from build123d import *

# Parameters (mm, degrees)
BASE_BLOCK_70X40X40_DEPTH        = 40
BOTTOM_SLOT_SKETCH_W             = 24
BOTTOM_SLOT_SKETCH_H             = 14
BOTTOM_SLOT_DEPTH                = 35
BOTTOM_SLOT_EXTENSION_SKETCH_W   = 24
BOTTOM_SLOT_EXTENSION_SKETCH_H   = 14
BOTTOM_SLOT_EXTENSION_DEPTH      = 35
TOP_CHANNEL_SKETCH_W             = 14
TOP_CHANNEL_SKETCH_H             = 10
TOP_CHANNEL_DEPTH                = 49
SIDE_STEP_CUT_A_DEPTH            = 67.520673478
SIDE_STEP_CUT_A_DEPTH_BACK       = 95
SIDE_STEP_CUT_A_SKETCH_W         = 15
SIDE_STEP_CUT_A_SKETCH_H         = 16
SIDE_STEP_CUT_B_SKETCH_W         = 15
SIDE_STEP_CUT_B_SKETCH_H         = 16
SIDE_STEP_CUT_B_DEPTH            = 95
RIB_A_SKETCH_W                   = 15
RIB_A_SKETCH_H                   = 5
RIB_A_DEPTH                      = 16
RIB_A_TRIM_DEPTH                 = 40
RIB_A_TRIM_DEPTH_BACK            = 52
THROUGH_HOLE_16_DEPTH            = 52
THROUGH_HOLE_16_DEPTH_BACK       = 52
THROUGH_HOLE_16_SKETCH_R         = 8
RIB_B_SKETCH_W                   = 15
RIB_B_SKETCH_H                   = 5
RIB_B_DEPTH                      = 16
RIB_B_TRIM_DEPTH                 = 16
FOOT_RELIEF_CUT_DEPTH            = 23
FOOT_RELIEF_CUT_DEPTH_BACK       = 23
FOOT_RELIEF_SKETCH_W             = 50
FOOT_RELIEF_SKETCH_H             = 10
FOOT_RELIEF_EXTENSION_DEPTH      = 23
FOOT_RELIEF_EXTENSION_DEPTH_BACK = 23
FOOT_RELIEF_EXTENSION_SKETCH_W   = 50
FOOT_RELIEF_EXTENSION_SKETCH_H   = 10


with BuildPart() as part:
    # Base Block Sketch → Base Block 70x40x40 (new body)
    with BuildSketch(Plane(origin=(0, 0, 0), x_dir=(1, 0, 0), z_dir=(0, 1, 0))):
        Polygon((0, -20), (0, 0), (0, 20), (-35, 20), (-35, -20), align=None)
        Polygon((0, 20), (0, 0), (0, -20), (35, -20), (35, 20), align=None)
    extrude(amount=BASE_BLOCK_70X40X40_DEPTH)

    # Bottom Slot Sketch → Bottom Slot (cut)
    with BuildSketch(Plane.ZY.offset(35)):
        with Locations((0, 7)):
            Rectangle(BOTTOM_SLOT_SKETCH_W, BOTTOM_SLOT_SKETCH_H)
    extrude(amount=-BOTTOM_SLOT_DEPTH, mode=Mode.SUBTRACT)

    # Bottom Slot Extension Sketch → Bottom Slot Extension (cut)
    with BuildSketch(Plane.ZY):
        with Locations((0, 7)):
            Rectangle(BOTTOM_SLOT_EXTENSION_SKETCH_W, BOTTOM_SLOT_EXTENSION_SKETCH_H)
    extrude(amount=-BOTTOM_SLOT_EXTENSION_DEPTH, mode=Mode.SUBTRACT)

    # Top Channel Sketch → Top Channel (cut)
    with BuildSketch(Plane.XY.offset(20)):
        with Locations((-7, 35)):
            Rectangle(TOP_CHANNEL_SKETCH_W, TOP_CHANNEL_SKETCH_H)
        with Locations((7, 35)):
            Rectangle(TOP_CHANNEL_SKETCH_W, TOP_CHANNEL_SKETCH_H)
    extrude(amount=-TOP_CHANNEL_DEPTH, mode=Mode.SUBTRACT)

    # Side Step Cut A Sketch → Side Step Cut A (cut, two sides: drawn at the far end of the back side and taken through both)
    with BuildSketch(Plane.XY.offset(20).offset(-SIDE_STEP_CUT_A_DEPTH_BACK)):
        with Locations((27.5, 32)):
            Rectangle(SIDE_STEP_CUT_A_SKETCH_W, SIDE_STEP_CUT_A_SKETCH_H)
    extrude(amount=SIDE_STEP_CUT_A_DEPTH + SIDE_STEP_CUT_A_DEPTH_BACK, mode=Mode.SUBTRACT)

    # Side Step Cut B Sketch → Side Step Cut B (cut)
    with BuildSketch(Plane.XY.offset(20)):
        with Locations((-27.5, 32)):
            Rectangle(SIDE_STEP_CUT_B_SKETCH_W, SIDE_STEP_CUT_B_SKETCH_H)
    extrude(amount=-SIDE_STEP_CUT_B_DEPTH, mode=Mode.SUBTRACT)

    # Rib A Sketch → Rib A (add)
    with BuildSketch(Plane(origin=(0, 24, 0), x_dir=(1, 0, 0), z_dir=(0, 1, 0))):
        with Locations((-27.5, -2.5)):
            Rectangle(RIB_A_SKETCH_W, RIB_A_SKETCH_H)
        with Locations((-27.5, 2.5)):
            Rectangle(RIB_A_SKETCH_W, RIB_A_SKETCH_H)
    extrude(amount=RIB_A_DEPTH)

    # Rib A Trim Sketch → Rib A Trim (cut, two sides: drawn at the far end of the back side and taken through both)
    with BuildSketch(Plane.XY.offset(5).offset(-RIB_A_TRIM_DEPTH_BACK)):
        Polygon((-20, 40), (-35, 24), (-35, 40), align=None)
    extrude(amount=RIB_A_TRIM_DEPTH + RIB_A_TRIM_DEPTH_BACK, mode=Mode.SUBTRACT)

    # Through Hole _16 Sketch → Through Hole _16 (cut, two sides: drawn at the far end of the back side and taken through both)
    with BuildSketch(Plane(origin=(0, 30, 0), x_dir=(1, 0, 0), z_dir=(0, 1, 0)).offset(-THROUGH_HOLE_16_DEPTH_BACK)):
        with Locations(Location((0, 0, 0), (0, 0, 270))):
            Circle(THROUGH_HOLE_16_SKETCH_R)
    extrude(amount=THROUGH_HOLE_16_DEPTH + THROUGH_HOLE_16_DEPTH_BACK, mode=Mode.SUBTRACT)

    # Rib B Sketch → Rib B (add)
    with BuildSketch(Plane(origin=(0, 24, 0), x_dir=(1, 0, 0), z_dir=(0, 1, 0))):
        with Locations((27.5, -2.5)):
            Rectangle(RIB_B_SKETCH_W, RIB_B_SKETCH_H)
        with Locations((27.5, 2.5)):
            Rectangle(RIB_B_SKETCH_W, RIB_B_SKETCH_H)
    extrude(amount=RIB_B_DEPTH)

    # Rib B Trim Sketch → Rib B Trim (cut)
    with BuildSketch(Plane(origin=(0, 0, -5), x_dir=(-1, 0, 0), z_dir=(0, 0, -1))):
        Polygon((-20, 40), (-35, 24), (-35, 40), align=None)
    extrude(amount=-RIB_B_TRIM_DEPTH, mode=Mode.SUBTRACT)

    # Foot Relief Sketch → Foot Relief Cut (cut, two sides: drawn at the far end of the back side and taken through both)
    with BuildSketch(Plane(origin=(0, 0, -20), x_dir=(-1, 0, 0), z_dir=(0, 0, -1)).offset(-FOOT_RELIEF_CUT_DEPTH_BACK)):
        with Locations((0, 5)):
            Rectangle(FOOT_RELIEF_SKETCH_W, FOOT_RELIEF_SKETCH_H)
    extrude(amount=FOOT_RELIEF_CUT_DEPTH + FOOT_RELIEF_CUT_DEPTH_BACK, mode=Mode.SUBTRACT)

    # Foot Relief Extension Sketch → Foot Relief Extension (cut, two sides: drawn at the far end of the back side and taken through both)
    with BuildSketch(Plane(origin=(0, 0, 12), x_dir=(-1, 0, 0), z_dir=(0, 0, -1)).offset(-FOOT_RELIEF_EXTENSION_DEPTH_BACK)):
        with Locations((0, 5)):
            Rectangle(FOOT_RELIEF_EXTENSION_SKETCH_W, FOOT_RELIEF_EXTENSION_SKETCH_H)
    extrude(amount=FOOT_RELIEF_EXTENSION_DEPTH + FOOT_RELIEF_EXTENSION_DEPTH_BACK, mode=Mode.SUBTRACT)


solid = part.part
Input: part model. Units: mm. Frame: model coordinates. A direction names the side the tool comes from. Round coordinates to 2 decimals unless told otherwise and drop trailing zeros. Loops run counter-clockwise (first coordinate to the right, second up) from the corner with the lowest first, then second, coordinate; pieces in that order, holes last. Notation, with made-up numbers: (11, 37) -> (24, 37) arc R21 cw to (24, 69) -> close; hole circle Ø9 at (64.5, 9). An arc over 180 degrees is marked (long way). Answer as a JSON object with one key per item and string values. Group by question number.
1) Reachability of faces 4 (the flat face through (0, 12, 12)), 5 (the flat face through (-28, 24, -12)), 6 (the flat face through (-20, 32, 13)), 7 (the flat face through (-25, 5, -16)) from +Z, -Z, +X, -X, +Y, -Y: full face, straight path, thin tool, end or side. Return the list, or none.
2) Section query A-A on y = 8. Output: boundary loops of the cut face in (x, z).
3) Section query C-C on x = 0. Output: boundary loops of the cut face in (y, z).
4) Section query D-D on y = 27. Output: boundary loops of the cut face in (x, z), plus the area to 3 significant figures.
5) Section query B-B on z = 0. Output: boundary loops of the cut face in (x, y).
6) Pin query (flat end, axial travel): pin 1 (7.5 mm diameter, centred on x = 29.5, y = 34.5, fed in from -Z); pin 2 (6.5 mm diameter, centred on x = -3.5, z = 15.5, fed in from -Y); pin 3 (4 mm diameter, centred on x = 27.5, y = 34.5, fed in from +Z). Return the tip coordinate at first contact, or that it passes through.
7) Draft query along Z for faces 1 (the flat face through (-28, 24, 13)), 2 (the cylindrical face through (-7.81, 21.89, -1.73)), 3 (the flat face through (0, 20, 20)). Return one class per face: +Z half, -Z half, draft (parallel to the pull), parting line (faces both ways), or undercut.
8) Ray query, L1, parallel to X at y = 22.75, z = 0; L2, parallel to Z at x = -31, y = 6; L3, parallel to Z at x = 0, y = 20. Return the intervals inside material, ascending.
Reply:
{
 "1": {"face 4": "+X, -X, -Y", "face 5": "-Z, -X, +Y", "face 6": "+Z, -X, +Y", "face 7": "+Z, -Z, -Y"},
 "2": {"outline": "(-35, -20) -> (-25, -20) -> (-25, -12) -> (-35, -12) -> close; (-35, 12) -> (-25, 12) -> (-25, 20) -> (-35, 20) -> close; (25, -20) -> (35, -20) -> (35, -12) -> (25, -12) -> close; (25, 12) -> (35, 12) -> (35, 20) -> (25, 20) -> close"},
 "3": {"outline": "(10, -20) -> (30, -20) -> (30, -8) -> (14, -8) -> (14, -12) -> (10, -12) -> close; (10, 12) -> (14, 12) -> (14, 8) -> (30, 8) -> (30, 20) -> (10, 20) -> close"},
 "4": {"outline": "(-32.19, -5) -> (-20, -5) -> (-20, -20) -> (20, -20) -> (20, -5) -> (32.19, -5) -> (32.19, 5) -> (20, 5) -> (20, 20) -> (-20, 20) -> (-20, 5) -> (-32.19, 5) -> close; hole circle Ø16 at (0, 0)", "area": "1,640 mm2"},
 "5": {"outline": "(-35, 14) -> (-8, 14) -> (-8, 30) -> (-14, 30) -> (-14, 40) -> (-20, 40) -> (-35, 24) -> close; (8, 14) -> (35, 14) -> (35, 24) -> (20, 40) -> (14, 40) -> (14, 30) -> (8, 30) -> close"},
 "6": {"pin 1": "stops at z = -5", "pin 2": "stops at y = 10", "pin 3": "stops at z = 5"},
 "7": {"face 1": "draft", "face 2": "undercut", "face 3": "+Z half"},
 "8": {"L1": "x = -35 to -8, 8 to 35", "L2": "z = -20 to -12, 12 to 20", "L3": "z = -20 to -8, 8 to 20"}
}
